Input: part model. Units: mm. Frame: model coordinates. A direction names the side the tool comes from. Coordinates: 2 decimals unless noted, no trailing zeros. Order: outer loops, then holes, each group sorted by start corner. A loop starts at its lowest first (then second) coordinate and runs counter-clockwise, first axis right, second up. Notation, with made-up numbers: (84, -22) -> (100, -22) arc R12 cw to (100, -5) -> close; hole circle Ø2 at (71, 24). An arc over 180 degrees is marked (long way). Answer as CSV lines item,"result".
from build123d import *

# Parameters (mm, degrees)
MEMBER_C_12_1_DEPTH = 160
SKETCH_2_W          = 100
SKETCH_2_H          = 100
CUT_EXTRUDE_1_DEPTH = 40
CUT_EXTRUDE_2_REACH = 208.903
SKETCH_3_R          = 10


with BuildPart() as part:
    # Sketch11 → Member C _ 12_1 (new body)
    with BuildSketch(Plane(origin=(0, 0, 0), x_dir=(0, 0, -1), z_dir=(1, 0, 0))):
        with BuildLine():
            Line((53, 120), (0, 120))
            Line((0, 120), (0, 0))
            Line((0, 0), (53, 0))
            Line((53, 0), (53, 2.451956213))
            ThreePointArc((53, 2.451956213), (51.844151715, 5.463043942), (48.970378085, 6.927304742))
            Line((48.970378085, 6.927304742), (13.559243831, 10.649164928))
            ThreePointArc((13.559243831, 10.649164928), (7.811696571, 13.577686529), (5.5, 19.599861986))
            Line((5.5, 19.599861986), (5.5, 100.400138014))
            ThreePointArc((5.5, 100.400138014), (7.811696571, 106.422313471), (13.559243831, 109.350835072))
            Line((13.559243831, 109.350835072), (48.970378085, 113.072695258))
            ThreePointArc((48.970378085, 113.072695258), (51.844151715, 114.536956058), (53, 117.548043787))
            Line((53, 117.548043787), (53, 120))
        make_face()
    extrude(amount=MEMBER_C_12_1_DEPTH)

    # 草图2 → 切除-拉伸1 (cut)
    with BuildSketch(Plane.XY):
        with Locations((140, 60)):
            Rectangle(SKETCH_2_W, SKETCH_2_H)
    extrude(amount=-CUT_EXTRUDE_1_DEPTH, mode=Mode.SUBTRACT)

    # 切除-拉伸2: up to this face of the body (flat: up to its plane)
    cut_extrude_2_end = Plane(part.part.faces().sort_by_distance((80, 120, -26.5))[0])
    # 草图3 → 切除-拉伸2 (cut, up to the picked face)
    with BuildSketch(Plane.XZ, mode=Mode.PRIVATE) as cut_extrude_2_sk1:
        with Locations(Location((140, -33, 0), (0, 0, 270))):
            Circle(SKETCH_3_R)
    cut_extrude_2_tool1 = split(extrude(cut_extrude_2_sk1.sketch, amount=-CUT_EXTRUDE_2_REACH, mode=Mode.PRIVATE), bisect_by=cut_extrude_2_end, keep=Keep.BOTH, mode=Mode.PRIVATE)
    # 草图3 → 切除-拉伸2 (cut, up to the picked face)
    with BuildSketch(Plane.XZ, mode=Mode.PRIVATE) as cut_extrude_2_sk2:
        with Locations(Location((80, -33, 0), (0, 0, 270))):
            Circle(SKETCH_3_R)
    cut_extrude_2_tool2 = split(extrude(cut_extrude_2_sk2.sketch, amount=-CUT_EXTRUDE_2_REACH, mode=Mode.PRIVATE), bisect_by=cut_extrude_2_end, keep=Keep.BOTH, mode=Mode.PRIVATE)
    add(cut_extrude_2_tool1.solids().sort_by(Axis((140, 0, -33), (0, 1, 0)))[0], mode=Mode.SUBTRACT)
    add(cut_extrude_2_tool2.solids().sort_by(Axis((80, 0, -33), (0, 1, 0)))[0], mode=Mode.SUBTRACT)


solid = part.part
1. Cut plane D-D (x = 140). Return the cut outline in (y, z), plus the area to 3 significant figures.
Findings:
outline,"(0, -53) -> (2.45, -53) arc R4.5 ccw to (6.93, -48.97) -> (7.55, -43) -> (0, -43) -> close; (0, -23) -> (9.66, -23) -> (10, -19.74) -> (10, 0) -> (0, 0) -> close; (110, -19.74) -> (110.34, -23) -> (120, -23) -> (120, 0) -> (110, 0) -> close; (112.45, -43) -> (113.07, -48.97) arc R4.5 ccw to (117.55, -53) -> (120, -53) -> (120, -43) -> close"
area,"593 mm2"
2. Ray query, line 1 along X through (y, z) = (7.25, -33); line 2 along Y through (x, z) = (92, -20); line 3 along Z through (x, y) = (80, 116.25). Return the intervals inside material, ascending.
Findings:
line 1,"x = 0 to 70, 90 to 130, 150 to 160"
line 2,"y = 0 to 9.97, 110.03 to 120"
line 3,"z = -52.81 to -43, -23 to 0"
3. Cut plane C-C (y = 23). Return the cut outline in (x, z), plus the area to 3 significant figures.
Findings:
outline,"(0, -5.5) -> (90, -5.5) -> (90, 0) -> (0, 0) -> close"
area,"495 mm2"
4. Contact query for a flat-ended pin moving along its axis: pin 1 (6 mm diameter, centred on x = 130, z = -13.5, fed in from -Y). Output: stop coordinate, or through.
Findings:
pin 1,"stops at y = 0"
5. Cut plane A-A (z = -28). Return the cut outline in (x, y), plus the area to 3 significant figures.
Findings:
outline,"(0, 0) -> (71.34, 0) -> (71.34, 9.13) -> (0, 9.13) -> close; (0, 110.87) -> (71.34, 110.87) -> (71.34, 120) -> (0, 120) -> close; (88.66, 0) -> (131.34, 0) -> (131.34, 9.13) -> (88.66, 9.13) -> close; (88.66, 110.87) -> (131.34, 110.87) -> (131.34, 120) -> (88.66, 120) -> close; (148.66, 0) -> (160, 0) -> (160, 9.13) -> (148.66, 9.13) -> close; (148.66, 110.87) -> (160, 110.87) -> (160, 120) -> (148.66, 120) -> close"
area,"2,290 mm2"
6. Cut plane B-B (x = 80). Return the cut outline in (y, z).
Findings:
outline,"(0, -53) -> (2.45, -53) arc R4.5 ccw to (6.93, -48.97) -> (7.55, -43) -> (0, -43) -> close; (0, -23) -> (9.66, -23) -> (10.65, -13.56) arc R9 cw to (19.6, -5.5) -> (100.4, -5.5) arc R9 cw to (109.35, -13.56) -> (110.34, -23) -> (120, -23) -> (120, 0) -> (0, 0) -> close; (112.45, -43) -> (113.07, -48.97) arc R4.5 ccw to (117.55, -53) -> (120, -53) -> (120, -43) -> close"
7. Mould query, pull axis Y, two halves, no side actions, for faces 1 (the face through (79, 0, -20)), 2 (the face through (61, 61, 0)), 3 (the face through (125, 110, -10)), 4 (the face through (79, 120, -21)). Classes: released by +Y, released by -Y, zero draft, split by the parting line, or undercut.
Findings:
face 1,"released by -Y"
face 2,"zero draft"
face 3,"undercut"
face 4,"released by +Y"
8. Reachability of faces 5 (the face through (140, 5, -23)), 6 (the face through (44, 59, -5.5)), 7 (the face through (90, 60, -3)) from +Z, -Z, +X, -X, +Y, -Y: full face, straight path, thin tool, end or side. Return the list, or none.
Findings:
face 5,"+Y, -Y"
face 6,"-Z, +X, -X"
face 7,"+Z, -Z, +X"
